```python
from build123d import *

# Parameters (mm, degrees)
EXTRUDE_1_DEPTH             = 31
SKETCH_2_R                  = 1
CUT_EXTRUDE_1_DEPTH         = 104.997515993
FILLET_1_R                  = 10
FILLET_2_R                  = 20
FILLET_3_R                  = 5
HOLE_WIZARD_5_2_5_2_1_D     = 5.2
HOLE_WIZARD_5_2_5_2_1_DEPTH = 63
HOLE_WIZARD_5_2_5_2_1_TIP   = 1.562237609
HOLE_WIZARD_M6_1_D          = 5
HOLE_WIZARD_M6_1_DEPTH      = 8
HOLE_WIZARD_M6_1_TIP        = 1.502151548
SKETCH_7_R                  = 9.433771821
EXTRUDE_2_DEPTH             = 44


with BuildPart() as part:
    # 草图1 → 凸台-拉伸1 (new body)
    with BuildSketch(Plane(origin=(0, 0, 0), x_dir=(0, 0, -1), z_dir=(1, 0, 0))):
        Polygon((-55.379271635, 24.957586314), (14.620728365, 24.957586314), (14.620728365, -5.042413686), (-69.379271635, -5.042413686), (-69.379271635, -30.042413686), (40.620728365, -30.042413686), (40.620728365, 40.957586314), (-55.379271635, 40.957586314), align=None)
    extrude(amount=EXTRUDE_1_DEPTH)

    # 草图2 → 切除-拉伸1 (cut, through all)
    with BuildSketch(Plane(origin=(0, 40.957586314, 0), x_dir=(1, 0, 0), z_dir=(0, 1, 0))):
        with Locations(Location((15.5, -19.879271635, 0), (0, 0, 270))):
            Circle(SKETCH_2_R)
    extrude(amount=-CUT_EXTRUDE_1_DEPTH, mode=Mode.SUBTRACT)

    # 圆角1
    fillet_1_edges = [part.edges().sort_by_distance(p)[0] for p in [
        (15.5, 24.957586314, 55.379271635),
    ]]
    fillet(fillet_1_edges, radius=FILLET_1_R)

    # 圆角2
    fillet_2_edges = [part.edges().sort_by_distance(p)[0] for p in [
        (15.5, -5.042413686, 69.379271635),
    ]]
    fillet(fillet_2_edges, radius=FILLET_2_R)

    # 圆角3
    fillet_3_edges = [part.edges().sort_by_distance(p)[0] for p in [
        (15.5, -5.042413686, -14.620728365),
        (15.5, 24.957586314, -14.620728365),
    ]]
    fillet(fillet_3_edges, radius=FILLET_3_R)

    # Ø5.2 (5.2) 直径孔1
    with Locations(Plane(origin=(31, 0, 0), x_dir=(0, 0, -1), z_dir=(1, 0, 0))):
        with Locations((35.620728365, 30.957586314), (35.620728365, -1.042413686)):
            Hole(HOLE_WIZARD_5_2_5_2_1_D / 2, depth=HOLE_WIZARD_5_2_5_2_1_DEPTH)
            with Locations((0, 0, -(HOLE_WIZARD_5_2_5_2_1_DEPTH + HOLE_WIZARD_5_2_5_2_1_TIP / 2))):  # 118° drill point
                Cone(0, HOLE_WIZARD_5_2_5_2_1_D / 2, HOLE_WIZARD_5_2_5_2_1_TIP, mode=Mode.SUBTRACT)

    # M6 螺纹孔1
    with Locations(Plane(origin=(0, 0, -40.620728365), x_dir=(-1, 0, 0), z_dir=(0, 0, -1))):
        with Locations((-15.5, -13.042413686)):
            Hole(HOLE_WIZARD_M6_1_D / 2, depth=HOLE_WIZARD_M6_1_DEPTH)
            with Locations((0, 0, -(HOLE_WIZARD_M6_1_DEPTH + HOLE_WIZARD_M6_1_TIP / 2))):  # 118° drill point
                Cone(0, HOLE_WIZARD_M6_1_D / 2, HOLE_WIZARD_M6_1_TIP, mode=Mode.SUBTRACT)

    # 草图7 → 凸台-拉伸2 (add)
    with BuildSketch(Plane(origin=(0, 0, -40.620728365), x_dir=(-1, 0, 0), z_dir=(0, 0, -1))):
        with Locations(Location((-15.370770249, 16.377500271, 0), (0, 0, 180))):
            Circle(SKETCH_7_R)
    extrude(amount=EXTRUDE_2_DEPTH)


solid = part.part
```
The model under review builds one solid part; all positions refer to its coordinate system, in mm. A direction names the side the tool comes from. Round coordinates to 2 decimals unless told otherwise and drop trailing zeros. Loops run counter-clockwise (first coordinate to the right, second up) from the corner with the lowest first, then second, coordinate; pieces in that order, holes last.
Item 1: Take a section at A-A (z = -3). Write out the cut boundary in (x, y).
Determined:
outline: (0, -30.04) - (31, -30.04) - (31, -5.04) - (0, -5.04) - close; (0, 24.96) - (31, 24.96) - (31, 40.96) - (0, 40.96) - close
Item 2: For faces 4 (the face through (15.28, -0.93, -38.22)), 5 (the face through (15, 38, 55.379)), 6 (the face through (15, 24.958, 18)), 7 (the face through (8.42, 10, -62.31)), 8 (the face through (15, 16, -84.621)), list the 3-axis set-ups (+Z, -Z, +X, -X, +Y, -Y) from which the entire face can be reached by the end or side of a thin tool; tool diameter is ignored.
Determined:
face 4: +X, -X
face 5: +Z, +X, -X, +Y
face 6: +Z, +X, -X
face 7: -Z
face 8: -Z, +X, -X, +Y, -Y
Item 3: Take a section at D-D (y = 4.5). Write out the cut boundary in (x, z), then the cut area to 3 significant figures.
Determined:
outline: (0, -40.62) - (31, -40.62) - (31, -14.62) - (0, -14.62) - close
area: 806 mm2
Item 4: For line 1 (Y direction, x = 13.5, z = -1); line 2 (Y direction, x = 15, z = -36); line 3 (Y direction, x = 8, z = -37), list the stretches that pass through material, from the lowest coordinate up.
Determined:
line 1: y = -30.04 to -5.04, 24.96 to 40.96
line 2: y = -30.04 to -15.49, -10.59 to -3.61, 1.53 to 28.39, 33.53 to 40.96
line 3: y = -30.04 to -3.25, 1.16 to 28.75, 33.16 to 40.96
Item 5: Take a section at C-C (y = -7.5). Write out the cut boundary in (x, z).
Determined:
outline: (0, -40.62) - (31, -40.62) - (31, 58.98) - (0, 58.98) - close; hole circle Ø2 at (15.5, 19.88)
Item 6: Mouldability with a two-part tool opening along X and no side actions: class faces 1 (the face through (0, -10, 3)), 2 (the face through (13, -13, -37)), 3 (the face through (15.72, -10.75, 63.37)) as released by +X, released by -X, zero draft, split by the parting line, or undercut.
Determined:
face 1: released by -X
face 2: undercut
face 3: zero draft
Item 7: Clearance check with flat-ended pins moving along their axes: pin 1 Ø6.5 at (x, y) = (14, 36.5) entering from +Z; pin 2 Ø4 at (x, y) = (15.5, -13.04) entering from -Z; pin 3 Ø12 at (x, y) = (17, -19) entering from +Z; pin 4 Ø4 at (y, z) = (30.96, -35.62) entering from +X. State where each tip first meets the part, or that it passes through.
Determined:
pin 1: stops at z = 55.38
pin 2: stops at z = -32.32
pin 3: stops at z = 69.38
pin 4: passes through
Item 8: Take a section at B-B (x = 20). Write out the cut boundary in (y, z).
Determined:
outline: (-30.04, -40.62) - (8.16, -40.62) - (8.16, -84.62) - (24.6, -84.62) - (24.6, -40.62) - (40.96, -40.62) - (40.96, 55.38) - (34.96, 55.38) arc R10 ccw to (24.96, 45.38) - (24.96, -9.62) arc R5 cw to (19.96, -14.62) - (-0.04, -14.62) arc R5 cw to (-5.04, -9.62) - (-5.04, 49.38) arc R20 ccw to (-25.04, 69.38) - (-30.04, 69.38) - close; hole circle Ø5.2 at (-1.04, -35.62); hole circle Ø5.2 at (30.96, -35.62)
